The listing builds one solid part. Answer for the finished solid, in the listing's coordinates (mm). Face numbers are marked on the shaded views. A direction names the side the tool comes from. Coordinates: 2 decimals unless noted, no trailing zeros. Loops run counter-clockwise (first coordinate to the right, second up) from the corner with the lowest first, then second, coordinate; pieces in that order, holes last. Notation, with made-up numbers: (18, -13.5) - (69, -13.5) arc R36 cw to (69, 22.5) - close; hole circle Ø4 at (-9, 16). An arc over 180 degrees is marked (long way). Return JSON: item names as keys, results as strings. Group by question number.
1. Section C-C (z = -40.5) is taken. Write down the section's boundary in (x, y).
2. Each of these flat-tipped pins is pushed along its axis until it touches: P1, Ø19, axis at x = -3.5, z = -38.5, coming from the -Y side; P2, Ø5, axis at x = 4.5, z = -3, coming from the -Y side; P3, Ø2, axis at x = -17.5, y = -8.5, coming from the -Z side. Where does it stop, or does it pass through?
3. Find the intervals of material crossed by line 1 along Z through (x, y) = (100, -51); line 2 along Z through (x, y) = (-99, -12), in increasing order.
4. Section A-A (y = -65.5) is taken. Write down the section's boundary in (x, z).
5. Section D-D (x = 54.5) is taken. Write down the section's boundary in (y, z).
6. Section B-B (x = 14) is taken. Write down the section's boundary in (y, z).
7. Which of the six approach directions +Z, -Z, +X, -X, +Y, -Y give full straight-line access (tool end or side, diameter ignored) to the marked faces 1 and 2?
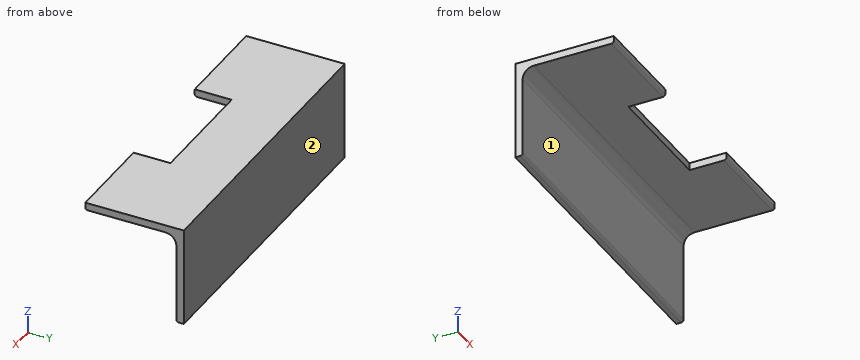
```python
from build123d import *

# Parameters (mm, degrees)
HOT_ROLLED_EQUAL_ANGLE_STEEL_GB_T_9787_DEPTH = 250
SKETCH3_W                                    = 95
SKETCH3_H                                    = 49.519926073
CUT_EXTRUDE1_DEPTH                           = 10


with BuildPart() as part:
    # Sketch1 → hot-rolled equal angle steel (GB/T 9787-1988) 80×6(1) (new body)
    with BuildSketch(Plane(origin=(125, 0, 0), x_dir=(0, -1, 0), z_dir=(-1, 0, 0))):
        with BuildLine():
            Line((80, 0), (0, 0))
            Line((0, 0), (0, -80))
            Line((0, -80), (4, -80))
            ThreePointArc((4, -80), (5.414213562, -79.414213562), (6, -78))
            Line((6, -78), (6, -15))
            ThreePointArc((6, -15), (8.636038969, -8.636038969), (15, -6))
            Line((15, -6), (78, -6))
            ThreePointArc((78, -6), (79.414213562, -5.414213562), (80, -4))
            Line((80, -4), (80, 0))
        make_face()
    extrude(amount=HOT_ROLLED_EQUAL_ANGLE_STEEL_GB_T_9787_DEPTH)

    # Sketch3 → Cut-Extrude1 (cut)
    with BuildSketch(Plane(origin=(0, 0, -6), x_dir=(-1, 0, 0), z_dir=(0, 0, -1))):
        with Locations((-2.5, -74.759963037)):
            Rectangle(SKETCH3_W, SKETCH3_H)
    extrude(amount=-CUT_EXTRUDE1_DEPTH, mode=Mode.SUBTRACT)


solid = part.part
```
The answers:
{
 "1": {"outline": "(-125, -6) - (125, -6) - (125, 0) - (-125, 0) - close"},
 "2": {"P1": "stops at y = -6", "P2": "stops at y = -50", "P3": "stops at z = -10.03"},
 "3": {"line 1": "z = -6 to 0", "line 2": "z = -6.51 to 0"},
 "4": {"outline": "(-125, -6) - (-45, -6) - (-45, 0) - (-125, 0) - close; (50, -6) - (125, -6) - (125, 0) - (50, 0) - close"},
 "5": {"outline": "(-80, -4) arc R2 ccw to (-78, -6) - (-15, -6) arc R9 cw to (-6, -15) - (-6, -78) arc R2 ccw to (-4, -80) - (0, -80) - (0, 0) - (-80, 0) - close"},
 "6": {"outline": "(-50, -6) - (-15, -6) arc R9 cw to (-6, -15) - (-6, -78) arc R2 ccw to (-4, -80) - (0, -80) - (0, 0) - (-50, 0) - close"},
 "7": {"face 1": "-Z, +X, -X, -Y", "face 2": "+Z, -Z, +X, -X, +Y"}
}
